```python
from build123d import *

# Parameters (mm, degrees)
BRACKET_BODY_DEPTH     = 19.05
FLANGE_HOLE_A_SKETCH_R = 6.35
FLANGE_HOLE_A_DEPTH    = 19.05
FLANGE_HOLE_B_SKETCH_R = 4.765
FLANGE_HOLE_B_DEPTH    = 19.05
BEND_FILLET_R1_63_A_R  = 1.63
BEND_FILLET_R1_63_B_R  = 1.63


with BuildPart() as part:
    # Bracket Profile Sketch → Bracket Body (new, symmetric)
    with BuildSketch(Plane.XY):
        with BuildLine():
            Line((0, 0), (44.59, 0))
            ThreePointArc((44.59, 0), (51.328727625, 2.791272375), (54.12, 9.53))
            Line((54.12, 9.53), (54.12, 85.72))
            ThreePointArc((54.12, 85.72), (51.328727625, 92.458727625), (44.59, 95.25))
            Line((44.59, 95.25), (-9.39, 95.25))
            Line((-9.39, 95.25), (-9.39, 88.9))
            Line((-9.39, 88.9), (47.77, 88.9))
            Line((47.77, 88.9), (47.77, 6.35))
            Line((47.77, 6.35), (2.311210988, 6.35))
            Line((2.311210988, 6.35), (-30.459242619, 33.847675535))
            Line((-30.459242619, 33.847675535), (-34.54094394, 28.983293321))
            Line((-34.54094394, 28.983293321), (0, 0))
        make_face()
    extrude(amount=BRACKET_BODY_DEPTH, both=True)

    # Flange Hole A Sketch → Flange Hole A (cut, symmetric)
    with BuildSketch(Plane(origin=(0, 95.25, 0), x_dir=(1, 0, 0), z_dir=(0, 1, 0))):
        with Locations(Location((9.65, 0, 0), (0, 0, 180))):
            Circle(FLANGE_HOLE_A_SKETCH_R)
    extrude(amount=FLANGE_HOLE_A_DEPTH, both=True, mode=Mode.SUBTRACT)

    # Flange Hole B Sketch → Flange Hole B (cut, symmetric)
    with BuildSketch(Plane(origin=(0, 0, 0), x_dir=(0.7660444431189771, -0.6427876096865404, 0), z_dir=(-0.6427876096865404, -0.7660444431189771, 0))):
        with Locations((-24.28, 0)):
            Circle(FLANGE_HOLE_B_SKETCH_R)
    extrude(amount=FLANGE_HOLE_B_DEPTH, both=True, mode=Mode.SUBTRACT)

    # Bend Fillet R1.63 A
    bend_fillet_r1_63_a_edges = [part.edges().sort_by_distance(p)[0] for p in [
        (47.77, 6.35, 0),
        (47.77, 88.9, 0),
    ]]
    fillet(bend_fillet_r1_63_a_edges, radius=BEND_FILLET_R1_63_A_R)

    # Bend Fillet R1.63 B
    bend_fillet_r1_63_b_edges = [part.edges().sort_by_distance(p)[0] for p in [
        (2.311210988, 6.35, 0),
    ]]
    fillet(bend_fillet_r1_63_b_edges, radius=BEND_FILLET_R1_63_B_R)


solid = part.part
```
Could you check a few things on this model? Use its own coordinates, in mm. A direction names the side the tool comes from. Coordinates: 2 decimals unless noted, no trailing zeros. Write each loop counter-clockwise with the first axis right and the second up, starting at its lowest first coordinate (ties: lowest second). Pieces come first, ordered by that corner, then holes. Notation, with made-up numbers: (40, -18) -> (86, -18) arc R23 cw to (86, 16) -> close; hole circle Ø11 at (82, 24). An arc over 180 degrees is marked (long way). Write item = value, one per line. Start each with the question number.
(1) Will these pins go through, and if not, where does the flat tip stop? pin 1 (5 mm diameter, centred on x = -20.5, z = 10.5, fed in from -Y); pin 2 (1.9 mm diameter, centred on y = 93, z = 4.5, fed in from -X); pin 3 (2 mm diameter, centred on x = -17, z = 15, fed in from +Y).
(2) I want a section at B-B (x = 34). Please give me the cut outline in (y, z), plus the area to 3 significant figures.
(3) I want a section at A-A (x = 9.65). Please give me the cut outline in (y, z).
(4) I want a section at C-C (z = -1.5). Please give me the cut outline in (x, y), plus the area to 3 significant figures.
(5) I want a section at D-D (z = -10). Please give me the cut outline in (x, y).
(6) We'd pull the mould along X, two halves only. Please class faces 1 (the face through (22, 0, 0)), 2 (the face through (-32.47, 31.45, 0.27)), 3 (the face through (54.12, 47, 0)), 4 (the face through (3.593, 92.119, 1.907)): released by +X, released by -X, zero draft, split by the parting line, or undercut.
(7) Which directions (+Z, -Z, +X, -X, +Y, -Y) give clear straight access to the entire face, cutting with the end or side of a thin tool? Please do faces 5 (the face through (-9.39, 92, 0)), 6 (the face through (18, 88.9, 0)), 7 (the face through (-10.5, 17.1, 0.3)).
(8) I need wall thicknesses on line 1 (Y direction, x = 3, z = 0.5); line 2 (X direction, y = 84.5, z = -2.5). Which ranges of each line are inside material? Lowest first, please. Write a range as [from, to].
Result set:
q1.pin_1 = 15.1
q1.pin_2 = -9.39
q1.pin_3 = 23.39
q2.outline = (0, -19.05) -> (6.35, -19.05) -> (6.35, 19.05) -> (0, 19.05) -> close; (88.9, -19.05) -> (95.25, -19.05) -> (95.25, 19.05) -> (88.9, 19.05) -> close
q2.area = 484 mm2
q3.outline = (0, -19.05) -> (6.35, -19.05) -> (6.35, 19.05) -> (0, 19.05) -> close; (88.9, -19.05) -> (95.25, -19.05) -> (95.25, -6.35) -> (88.9, -6.35) -> close; (88.9, 6.35) -> (95.25, 6.35) -> (95.25, 19.05) -> (88.9, 19.05) -> close
q4.outline = (-34.54, 28.98) -> (-22.06, 18.51) -> (-17.98, 23.38) -> (-30.46, 33.85) -> close; (-15.13, 12.7) -> (0, 0) -> (44.59, 0) arc R9.53 ccw to (54.12, 9.53) -> (54.12, 85.72) arc R9.53 ccw to (44.59, 95.25) -> (15.82, 95.25) -> (15.82, 88.9) -> (46.14, 88.9) arc R1.63 cw to (47.77, 87.27) -> (47.77, 7.98) arc R1.63 cw to (46.14, 6.35) -> (2.9, 6.35) arc R1.63 cw to (1.86, 6.73) -> (-11.05, 17.56) -> close; (-9.39, 88.9) -> (3.48, 88.9) -> (3.48, 95.25) -> (-9.39, 95.25) -> close
q4.area = 1,370 mm2
q5.outline = (-34.54, 28.98) -> (0, 0) -> (44.59, 0) arc R9.53 ccw to (54.12, 9.53) -> (54.12, 85.72) arc R9.53 ccw to (44.59, 95.25) -> (-9.39, 95.25) -> (-9.39, 88.9) -> (46.14, 88.9) arc R1.63 cw to (47.77, 87.27) -> (47.77, 7.98) arc R1.63 cw to (46.14, 6.35) -> (2.9, 6.35) arc R1.63 cw to (1.86, 6.73) -> (-30.46, 33.85) -> close
q6.face_1 = zero draft
q6.face_2 = released by -X
q6.face_3 = released by +X
q6.face_4 = undercut
q7.face_5 = +Z, -Z, -X, +Y
q7.face_6 = +Z, -Z, -X
q7.face_7 = +Z, -Z
q8.line_1 = [0, 6.35], [88.9, 95.25]
q8.line_2 = [47.77, 54.12]
